For this review, take the finished solid that the model builds, in its own axes (mm). A direction names the side the tool comes from. Give positions to 0.01 mm unless a question says otherwise; leave off trailing zeros. Write each loop counter-clockwise with the first axis right and the second up, starting at its lowest first coordinate (ties: lowest second). Pieces come first, ordered by that corner, then holes. Notation, with made-up numbers: M -39.75,50 L -0.75,50 A27 cw -0.75,86 Z; hole C 66.5,-33.75 d6. An arc over 180 degrees is marked long. Use one line per item in the form item = value. Start each with the question number.
Q1. Consider section A-A on z = 1.25. Write out the cut boundary in (x, y), and give its area (3 significant figures).
Q2. Mouldability with a two-part tool opening along X and no side actions: class faces 3 (the flat face through (28, 9.088, 5)), 4 (the cylindrical face through (51.94, -13.81, 5.8)), 5 (the cylindrical face through (28.334, -13.814, 6.278)), 6 (the flat face through (12, -5, 5)) as released by +X, released by -X, zero draft, split by the parting line, or undercut.
Q3. Tool access review of faces 1 (the cylindrical face through (19.1, -8.83, 5.27)), 2 (the flat face through (37, -6, 10)): name each direction out of +Z, -Z, +X, -X, +Y, -Y from which nothing blocks a thin tool from reaching the whole face with its end or side.
Q4. Consider section C-C on x = 45.5. Write out the cut boundary in (y, z).
Q5. For probe 1 along Y at (x, z) = (20.25, 5); probe 2 along Z at (x, y) = (50, -12); probe 3 along X at (y, z) = (-10, 6.25), list the stretches that pass through material, from the lowest coordinate up. Write a range as [from, to].
Q6. Clearance check with flat-ended pins moving along their axes: pin 1 Ø1 at (y, z) = (3, 5) entering from +X; pin 2 Ø3.5 at (x, z) = (50, 5) entering from -Y. State where each tip first meets the part, or that it passes through.
Q7. Consider section B-B on y = 5.75. Write out the cut boundary in (x, z), and give its area (3 significant figures).
```python
from build123d import *

# Parameters (mm, degrees)
EXTRUDE_1_DEPTH        = 10
CHAMFER_1_SIZE         = 2
HOLE_WIZARD_M5_1_D     = 4.2
HOLE_WIZARD_M5_1_DEPTH = 14
HOLE_WIZARD_M5_1_TIP   = 1.2618073
HOLE_WIZARD_M5_2_D     = 4.2
HOLE_WIZARD_M5_2_DEPTH = 14
HOLE_WIZARD_M5_2_TIP   = 1.2618073


with BuildPart() as part:
    # 草图1 → 凸台-拉伸1 (new body)
    with BuildSketch(Plane.XY):
        Polygon((62, -20.911504847), (12, -20.911504847), (12, 9.088495153), (44, 9.088495153), (62, -8.911504847), align=None)
    extrude(amount=EXTRUDE_1_DEPTH)

    # 倒角1
    chamfer_1_edges = [part.edges().sort_by_distance(p)[0] for p in [
        (12, -20.911504847, 5),
    ]]
    chamfer(chamfer_1_edges, length=CHAMFER_1_SIZE)

    # M5 螺纹孔1
    with Locations(Plane.ZY.offset(-12)):
        with Locations((5, -10.911504847), (5, 1.088495153)):
            Hole(HOLE_WIZARD_M5_1_D / 2, depth=HOLE_WIZARD_M5_1_DEPTH)
            with Locations((0, 0, -(HOLE_WIZARD_M5_1_DEPTH + HOLE_WIZARD_M5_1_TIP / 2))):  # 118° drill point
                Cone(0, HOLE_WIZARD_M5_1_D / 2, HOLE_WIZARD_M5_1_TIP, mode=Mode.SUBTRACT)

    # M5 螺纹孔2
    with Locations(Plane(origin=(0, -20.911504847, 0), x_dir=(-1, 0, 0), z_dir=(0, -1, 0))):
        with Locations((-30, -5), (-50, -5)):
            Hole(HOLE_WIZARD_M5_2_D / 2, depth=HOLE_WIZARD_M5_2_DEPTH)
            with Locations((0, 0, -(HOLE_WIZARD_M5_2_DEPTH + HOLE_WIZARD_M5_2_TIP / 2))):  # 118° drill point
                Cone(0, HOLE_WIZARD_M5_2_D / 2, HOLE_WIZARD_M5_2_TIP, mode=Mode.SUBTRACT)


solid = part.part
```
Working result:
q1.outline = M 12,-18.91 L 14,-20.91 L 62,-20.91 L 62,-8.91 L 44,9.09 L 12,9.09 Z
q1.area = 1,340 mm²
q2.face_3 = zero draft
q2.face_4 = undercut
q2.face_5 = undercut
q2.face_6 = released by -X
q3.face_1 = -X
q3.face_2 = +Z, +X, -X, +Y, -Y
q4.outline = M -20.91,0 L 7.59,0 L 7.59,10 L -20.91,10 Z
q5.probe_1 = [-20.91, -13.01], [-8.81, -1.01], [3.19, 9.09]
q5.probe_2 = [0, 2.9], [7.1, 10]
q5.probe_3 = [26.33, 28.31], [31.69, 48.31], [51.69, 62]
q6.pin_1 = 50.59
q6.pin_2 = -6.7
q7.outline = M 12,0 L 47.34,0 L 47.34,10 L 12,10 Z
q7.area = 353 mm²
